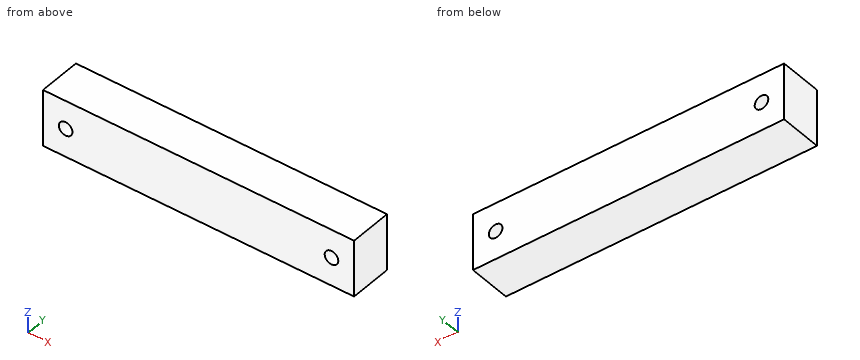
```python
from build123d import *

# Parameters (mm, degrees)
SKETCH_1_W         = 110
SKETCH_1_H         = 20
EXTRUDE_1_DEPTH    = 15
HOLE_WIZARD_M4_1_D = 4.8


with BuildPart() as part:
    # 草图1 → 凸台-拉伸1 (new body)
    with BuildSketch(Plane(origin=(0, 0, 0), x_dir=(1, 0, 0), z_dir=(0, 1, 0))):
        Rectangle(SKETCH_1_W, SKETCH_1_H)
    extrude(amount=EXTRUDE_1_DEPTH)

    # M4 间隙孔1 (through all)
    with Locations(Plane(origin=(0, 15, 0), x_dir=(1, 0, 0), z_dir=(0, 1, 0))):
        with Locations((-47, 0), (47, 0)):
            Hole(HOLE_WIZARD_M4_1_D / 2)


solid = part.part
```
Part model, mm, in its own coordinate system. Round coordinates to 2 decimals unless told otherwise and drop trailing zeros. Loops run counter-clockwise (first coordinate to the right, second up) from the corner with the lowest first, then second, coordinate; pieces in that order, holes last.
1. Slice it at A-A (z = 0). Give the cut face in (x, y), and give its area (3 significant figures).
Solutions:
outline: (-55, 0) - (-49.4, 0) - (-49.4, 15) - (-55, 15) - close; (-44.6, 0) - (44.6, 0) - (44.6, 15) - (-44.6, 15) - close; (49.4, 0) - (55, 0) - (55, 15) - (49.4, 15) - close
area: 1,510 mm2
2. Slice it at B-B (x = -47). Give the cut face in (y, z).
Solutions:
outline: (0, -10) - (15, -10) - (15, -2.4) - (0, -2.4) - close; (0, 2.4) - (15, 2.4) - (15, 10) - (0, 10) - close
3. Flat gauge pin, fed straight in: pin 1 (4.5 mm diameter, centred on x = -47, z = 0, fed in from -Y). Where does the tip first touch, or does it go through?
Solutions:
pin 1: passes through
4. Slice it at C-C (y = 3.5). Give the cut face in (x, z).
Solutions:
outline: (-55, -10) - (55, -10) - (55, 10) - (-55, 10) - close; hole circle Ø4.8 at (-47, 0); hole circle Ø4.8 at (47, 0)
5. Drill centre lines: line 1 along Z through (x, y) = (-47, 10); line 2 along X through (y, z) = (14, 0.75); line 3 along Z through (x, y) = (-49, 14.25). Where is each one in solid material? Low to high.
Solutions:
line 1: z = -10 to -2.4, 2.4 to 10
line 2: x = -55 to -49.28, -44.72 to 44.72, 49.28 to 55
line 3: z = -10 to -1.33, 1.33 to 10
